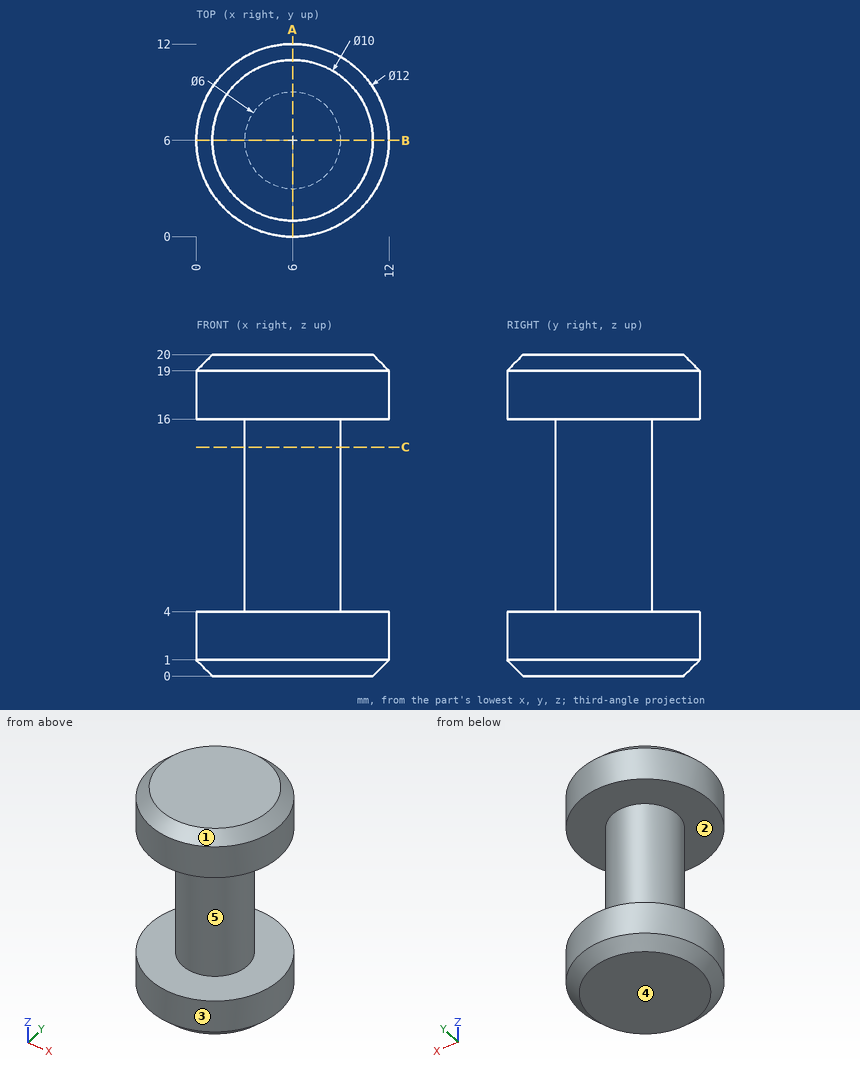
Geometry check sheet. Reference: drawing and pictorial views, mm from the part's lowest x, y, z. A direction names the side the tool comes from. Round coordinates to 2 decimals unless told otherwise and drop trailing zeros. Write each loop counter-clockwise with the first axis right and the second up, starting at its lowest first coordinate (ties: lowest second). Pieces come first, ordered by that corner, then holes.
Item 1: Material ranges on line 1 along Z through (x, y) = (1.25, 6.25); line 2 along Y through (x, z) = (6, 7.75); line 3 along Z through (x, y) = (11, 9.25), recorded low to high.
Determined:
line 1: z = 0 to 4, 16 to 20
line 2: y = 3 to 9
line 3: z = 0.96 to 4, 16 to 19.04
Item 2: Mould release check, pull along Z, two halves, no side actions. Record for the marked faces 1, 2 and 3: +Z half, -Z half, draft (parallel to the pull), parting line (faces both ways), or undercut.
Determined:
face 1: +Z half
face 2: undercut
face 3: draft
Item 3: Go/stop test with flat-tipped pins: pin 1 Ø1 at (x, z) = (6.5, 10) entering from +Y; pin 2 Ø3 at (x, z) = (8.5, 7) entering from +Y; pin 3 Ø5 at (y, z) = (10.5, 8) entering from -X. Record where each tip stops, or that it passes through.
Determined:
pin 1: stops at y = 9
pin 2: stops at y = 8.83
pin 3: stops at x = 3.76
Item 4: Section check C-C (z = 14.25). Record the boundary of the cut face in (x, y), plus the area to 3 significant figures.
Determined:
outline: circle Ø6 at (6, 6)
area: 28.3 mm2
Item 5: Access from +Z, -Z, +X, -X, +Y, -Y to the whole of each face (thin tool, end or side, straight path). Record for the marked faces 4 and 5.
Determined:
face 4: -Z, +X, -X, +Y, -Y
face 5: none
Item 6: Section check A-A (x = 6). Record the boundary of the cut face in (y, z), plus the area to 3 significant figures.
Determined:
outline: (0, 1) - (1, 0) - (11, 0) - (12, 1) - (12, 4) - (9, 4) - (9, 16) - (12, 16) - (12, 19) - (11, 20) - (1, 20) - (0, 19) - (0, 16) - (3, 16) - (3, 4) - (0, 4) - close
area: 166 mm2
